from build123d import *

# Parameters (mm, degrees)
EXTRUDE_START   = -6
SKETCH_2_R      = 27
SKETCH_2_R_2    = 21.5
EXTRUDE_1_DEPTH = 7


with BuildPart() as part:
    # 草图1 → 旋转1 (revolve)
    with BuildSketch(Plane.XY, mode=Mode.PRIVATE) as revolve_1_sk:
        Polygon((0, 13), (0, 20), (125, 20), (125, 21.5), (147, 21.5), (147, 13), align=None)
    revolve(revolve_1_sk.sketch.rotate(Axis((0, 0, 0), (1, 0, 0)), 90), axis=Axis((0, 0, 0), (1, 0, 0)))

    # 草图2 → 凸台-拉伸1 (add)
    with BuildSketch(Plane(origin=(147, 0, 0), x_dir=(0, 0, -1), z_dir=(1, 0, 0)).offset(EXTRUDE_START)):
        Circle(SKETCH_2_R)
        with Locations(Location((0, 0, 0), (0, 0, 180))):
            Circle(SKETCH_2_R_2, mode=Mode.SUBTRACT)
    extrude(amount=-EXTRUDE_1_DEPTH)


solid = part.part
Model file for the job. Use its own axes, mm. A direction names the side the tool comes from. Round coordinates to 2 decimals unless told otherwise and drop trailing zeros. Order: outer loops, then holes, each group sorted by start corner. A loop starts at its lowest first (then second) coordinate and runs counter-clockwise, first axis right, second up.
(1) Drill centre lines: line 1 (Y direction, x = 39, z = 0); line 2 (X direction, y = -21.5, z = -3); line 3 (Y direction, x = 86, z = -11). Where is each one in solid material? Low to high.
(2) Pin check, flat tips, straight feed: pin 1 (2 mm diameter, centred on x = 81, y = -13, fed in from -Z); pin 2 (8 mm diameter, centred on x = 62, y = 16.5, fed in from +Z); pin 3 (1 mm diameter, centred on x = 41.5, z = 7.5, fed in from -Y) (3 decimals); pin 4 (21 mm diameter, centred on y = 0, z = 0, fed in from -X). Stop position of each tip, or through.
(3) 3-axis set-ups, long thin cutter, end or side, ignore diameter. For faces 1 (the face through (141, -11.9, 18.1)), 2 (the face through (63.38, -0.88, -19.98)), 3 (the face through (137.55, -26.36, 5.85)): which of +Z, -Z, +X, -X, +Y, -Y reach the whole face in a straight line?
(4) Band-saw the part on C-C (x = 74). List the corners of the cut face in (y, z).
(5) Band-saw the part on D-D (y = 24.5). List the corners of the cut face in (x, z), then the cut area to 3 significant figures.
(6) Pull direction Z, two halves, no side cores. Call faces 4 (the face through (72.471, 7.91, -10.316)), 5 (the face through (0, 13, -4)), 6 (the face through (129.563, -21.317, -2.799)): released by +Z, released by -Z, zero draft, split by the parting line, or undercut.
(7) Band-saw the part on A-A (z = 0). List the corners of the cut face in (x, y).
Verdict:
1. line 1: y = -20 to -13, 13 to 20
1. line 2: x = 134 to 141
1. line 3: y = -16.7 to -6.93, 6.93 to 16.7
2. pin 1: stops at z = -16
2. pin 2: stops at z = 15.61
2. pin 3: stops at y = -18.735
2. pin 4: passes through
3. face 1: +X
3. face 2: -X
3. face 3: +X, -X
4. outline: circle Ø40 at (0, 0); hole circle Ø26 at (0, 0)
5. outline: (134, -11.35) - (141, -11.35) - (141, 11.35) - (134, 11.35) - close
5. area: 159 mm2
6. face 4: undercut
6. face 5: zero draft
6. face 6: split by the parting line
7. outline: (0, -20) - (125, -20) - (125, -21.5) - (134, -21.5) - (134, -27) - (141, -27) - (141, -21.5) - (147, -21.5) - (147, -13) - (0, -13) - close; (0, 13) - (147, 13) - (147, 21.5) - (141, 21.5) - (141, 27) - (134, 27) - (134, 21.5) - (125, 21.5) - (125, 20) - (0, 20) - close
